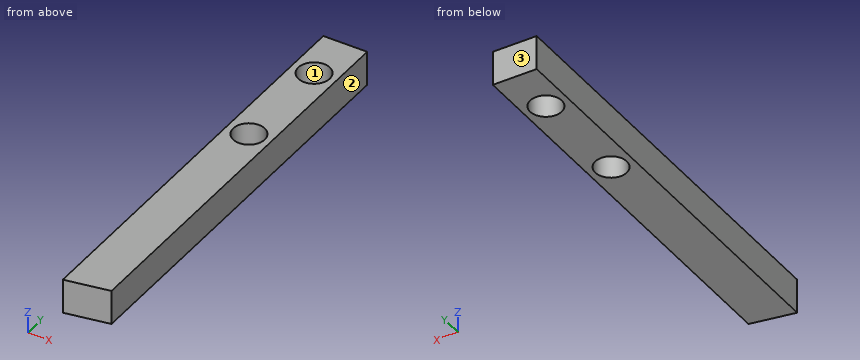
```python
from build123d import *

# Parameters (mm, degrees)
SKETCH1_W           = 4.18
SKETCH1_H           = 3.28
BOSS_EXTRUDE1_DEPTH = 40
CUT_EXTRUDE1_DEPTH  = 40
SKETCH3_R           = 1.5
CUT_EXTRUDE2_DEPTH  = 40


with BuildPart() as part:
    # Sketch1 → Boss-Extrude1 (new body)
    with BuildSketch(Plane(origin=(0, 0, 0), x_dir=(1, 0, 0), z_dir=(0, 1, 0))):
        Rectangle(SKETCH1_W, SKETCH1_H)
    extrude(amount=BOSS_EXTRUDE1_DEPTH)

    # Sketch2 → Cut-Extrude1 (cut)
    with BuildSketch(Plane.XY.offset(1.64)):
        Polygon((-2.09, 0), (2.09, 0), (2.09, 0.737046779), align=None)
    extrude(amount=-CUT_EXTRUDE1_DEPTH, mode=Mode.SUBTRACT)

    # Sketch3 → Cut-Extrude2 (cut)
    with BuildSketch(Plane(origin=(0, 0, -1.64), x_dir=(-1, 0, 0), z_dir=(0, 0, -1))):
        with Locations((0, 35.211206118)):
            Circle(SKETCH3_R)
        with Locations((0, 25.211206118)):
            Circle(SKETCH3_R)
    extrude(amount=-CUT_EXTRUDE2_DEPTH, mode=Mode.SUBTRACT)


solid = part.part
```
Here's how the part is built. I have some questions about the finished solid (model axes, mm). Face numbers are marked on the shaded views. Round coordinates to 2 decimals unless told otherwise and drop trailing zeros. Write each loop counter-clockwise with the first axis right and the second up, starting at its lowest first coordinate (ties: lowest second). Pieces come first, ordered by that corner, then holes.
Q1. Will this pin go through, and if not, where does the flat tip stop? P1, Ø1.8, axis at x = 0, y = 25.21, coming from the +Z side.
Q2. If we section it at B-B on z = -0.55: Write out the boundary of the cut face in (x, y), plus the area to 3 significant figures.
Q3. Please list where these lines run through material, in increasing order: probe 1 along Y at (x, z) = (0, -0.2); probe 2 along Y at (x, z) = (1.3, -0.6); probe 3 along X at (y, z) = (36.5, -0.05).
Q4. If we section it at A-A on x = 0.25: Write out the boundary of the cut face in (y, z).
Q5. If we mould it in two halves opening along X, with no side actions, what happens to the marked faces 1, 2 and 3? For each: +X half, -X half, draft (parallel to the pull), parting line (faces both ways), or undercut.
Answer below:
1. P1: passes through
2. outline: (-2.09, 0) - (2.09, 0.74) - (2.09, 40) - (-2.09, 40) - close; hole circle Ø3 at (0, 25.21); hole circle Ø3 at (0, 35.21)
2. area: 152 mm2
3. probe 1: y = 0.37 to 23.71, 26.71 to 33.71, 36.71 to 40
3. probe 2: y = 0.6 to 24.46, 25.96 to 34.46, 35.96 to 40
3. probe 3: x = -2.09 to -0.77, 0.77 to 2.09
4. outline: (0.41, -1.64) - (23.73, -1.64) - (23.73, 1.64) - (0.41, 1.64) - close; (26.69, -1.64) - (33.73, -1.64) - (33.73, 1.64) - (26.69, 1.64) - close; (36.69, -1.64) - (40, -1.64) - (40, 1.64) - (36.69, 1.64) - close
5. face 1: undercut
5. face 2: +X half
5. face 3: draft
